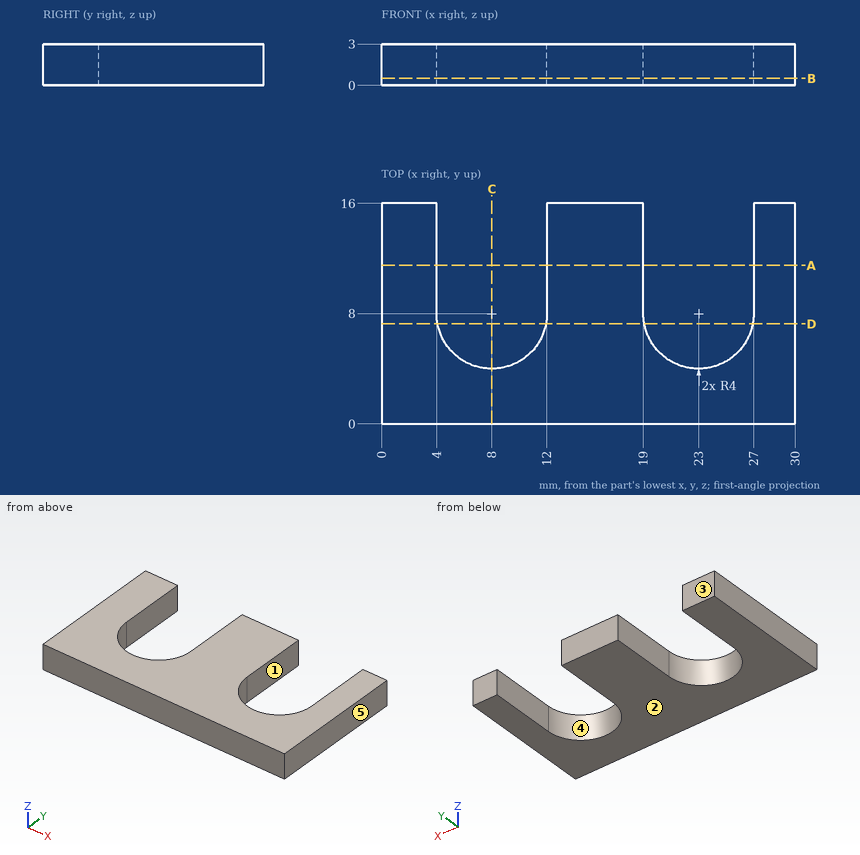
Input: dimensioned drawing with shaded views. Units: mm. Origin: part minimum x, y, z. A direction names the side the tool comes from. Coordinates: 2 decimals unless noted, no trailing zeros. Loops run counter-clockwise (first coordinate to the right, second up) from the corner with the lowest first, then second, coordinate; pieces in that order, holes last. Notation, with made-up numbers: M -20,73.25 L -16,73.25 A23 ccw -16,110.25 Z; hole C 60.25,7.25 d5. An arc over 180 degrees is marked long. One line per item, written item: value. Start each with the question number.
1) Draft query along X for the marked faces 3, 4 and 5. Return one class per face: released by +X, released by -X, zero draft, split by the parting line, or undercut.
2) Material intervals for L1, parallel to X at y = 10.25, z = 1.6; L2, parallel to X at y = 4.5, z = 2.6; L3, parallel to Y at x = 20.75, z = 0.75, sorted ascending. Write a range as from..to.
3) Cut plane D-D (y = 7.25). Return loops of the section in (x, z), then the cut area to 3 significant figures.
4) Cut plane B-B (z = 0.5). Return loops of the section in (x, y).
5) Cut plane A-A (y = 11.5). Return loops of the section in (x, z).
6) Pin query (flat end, axial travel): P1, Ø1.5, axis at x = 13, y = 12.5, coming from the -Z side; P2, Ø2, axis at x = 9, y = 5.5, coming from the -Z side. Return the tip coordinate at first contact, or that it passes through.
7) Cut plane C-C (x = 8). Return loops of the section in (y, z).
8) Reachability of the marked faces 1 and 2 from +Z, -Z, +X, -X, +Y, -Y: full face, straight path, thin tool, end or side. Return the list, or none.
Evaluation:
1. face 3: zero draft
1. face 4: undercut
1. face 5: released by +X
2. L1: 0..4, 12..19, 27..30
2. L2: 0..6.06, 9.94..21.06, 24.94..30
2. L3: 0..4.69
3. outline: M 0,0 L 4.07,0 L 4.07,3 L 0,3 Z; M 11.93,0 L 19.07,0 L 19.07,3 L 11.93,3 Z; M 26.93,0 L 30,0 L 30,3 L 26.93,3 Z
3. area: 42.9 mm^2
4. outline: M 0,0 L 30,0 L 30,16 L 27,16 L 27,8 A4 cw 19,8 L 19,16 L 12,16 L 12,8 A4 cw 4,8 L 4,16 L 0,16 Z
5. outline: M 0,0 L 4,0 L 4,3 L 0,3 Z; M 12,0 L 19,0 L 19,3 L 12,3 Z; M 27,0 L 30,0 L 30,3 L 27,3 Z
6. P1: z = 0
6. P2: through
7. outline: M 0,0 L 4,0 L 4,3 L 0,3 Z
8. face 1: +Z, -Z, +Y
8. face 2: -Z, +X, -X, +Y, -Y
